from build123d import *

# Parameters (mm, degrees)
FILLET1_R = 80
SHELL1_T  = -70


with BuildPart() as part:
    # Sketch2 → Revolve1 (revolve)
    with BuildSketch(Plane.XY, mode=Mode.PRIVATE) as revolve1_sk:
        Polygon((0, 1700), (250, 1700), (250, 300), (80, 0), (0, 0), align=None)
    revolve(revolve1_sk.sketch.rotate(Axis((0, 0, 0), (0, 1, 0)), 270), axis=Axis((0, 0, 0), (0, 1, 0)))

    # Fillet1
    fillet1_edges = [part.edges().sort_by_distance(p)[0] for p in [
        (0, 0, -80),
    ]]
    fillet(fillet1_edges, radius=FILLET1_R)

    # Shell1
    shell1_openings = [part.faces().sort_by_distance(p)[0] for p in [
        (0, 1700, 0),
    ]]
    offset(amount=SHELL1_T, openings=shell1_openings, kind=Kind.INTERSECTION)


solid = part.part
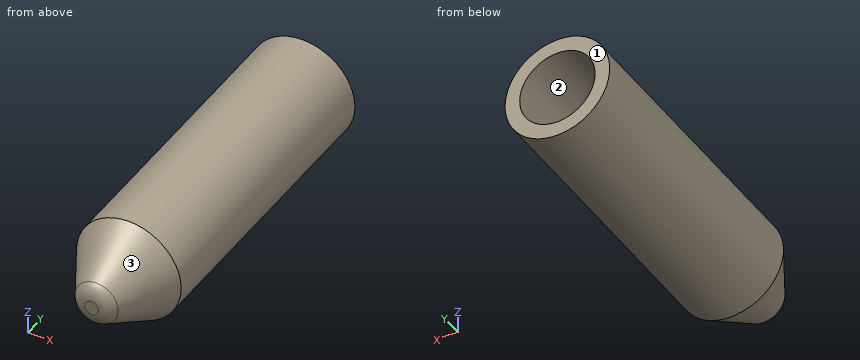
Could you check a few things on this model? Use its own coordinates, in mm. Face numbers are marked on the shaded views. Give positions to 0.01 mm unless a question says otherwise; leave off trailing zeros. Order: outer loops, then holes, each group sorted by start corner. A loop starts at its lowest first (then second) coordinate and runs counter-clockwise, first axis right, second up. Notation, with made-up numbers: M -36.75,-26 L -27.75,-26 A12 ccw -27.75,-5 Z; hole C -25,73.5 d11. An arc over 180 degrees is marked long. One line per question, with ' | ' between items.
1. If I drill on line 1 (X direction, y = 823, z = 0); line 2 (X direction, y = 1453, z = -37); line 3 (Z direction, x = 67, y = 1351), over which ranges is the centre line in solid material (lowest first)?
Results:
line 1: -250 to -180, 180 to 250 | line 2: -247.25 to -176.16, 176.16 to 247.25 | line 3: -240.85 to -167.07, 167.07 to 240.85
2. I'm going to push flat-ended pins straight in: pin 1 (4 mm diameter, centred on y = 311.5, z = 161, fed in from -X); pin 2 (2 mm diameter, centred on y = 1472.5, z = 109, fed in from +X); pin 3 (12 mm diameter, centred on x = -149.5, y = 1121, fed in from +Z). Where does each tip first touch, or does it pass through?
Results:
pin 1: x = -192.92 | pin 2: x = 225.47 | pin 3: z = 204.71
3. We'd pull the mould along X, two halves only. Please class the marked faces 1, 2 and 3: +X half, -X half, draft (parallel to the pull), parting line (faces both ways), or undercut.
Results:
face 1: draft | face 2: undercut | face 3: parting line
4. I want a section at A-A (y = 129.5). List the corners of the cut face in (x, z) for me, and give its area (3 significant figures).
Results:
outline: C 0,0 d306.77; hole C 0,0 d145.85 | area: 57,200 mm²
